```python
from build123d import *

# Parameters (mm, degrees)
SKETCH4_W          = 1.2
SKETCH4_H          = 1.2
CUT_EXTRUDE1_DEPTH = 50


with BuildPart() as part:
    # Sketch3 → Boss-Revolve (revolve)
    with BuildSketch(Plane.XY, mode=Mode.PRIVATE) as boss_revolve_sk:
        with BuildLine():
            Line((0, 0), (15, 0))
            Line((15, 0), (15, 2.5))
            Line((15, 2.5), (4.6, 2.5))
            Line((4.6, 2.5), (4.265, 2.165))
            Line((4.265, 2.165), (3.685, 2.165))
            ThreePointArc((3.685, 2.165), (3.200631855, 2.365631855), (3, 2.85))
            Line((3, 2.85), (3, 4.75))
            Line((3, 4.75), (1.369266386, 4.607329296))
            ThreePointArc((1.369266386, 4.607329296), (0.394083995, 4.12642256), (0, 3.113037248))
            Line((0, 3.113037248), (0, 0))
        make_face()
    revolve(boss_revolve_sk.sketch.rotate(Axis((-2.477021524, 0, 0), (1, 0, 0)), 90), axis=Axis((-2.477021524, 0, 0), (1, 0, 0)))

    # Sketch4 → Cut-Extrude1 (cut, symmetric)
    with BuildSketch(Plane.XY):
        with Locations((0.6, 0)):
            Rectangle(SKETCH4_W, SKETCH4_H)
    extrude(amount=CUT_EXTRUDE1_DEPTH, both=True, mode=Mode.SUBTRACT)

    # Sketch5 → Cut-Revolve1 (revolve, cut)
    with BuildSketch(Plane.XY, mode=Mode.PRIVATE) as cut_revolve1_sk:
        Polygon((14.595667195, 2.5), (15.395667195, 2.5), (15, 1.8072), align=None)
    revolve(cut_revolve1_sk.sketch.rotate(Axis((6.174994867, 0, 0), (-1, 0, 0)), 270), axis=Axis((6.174994867, 0, 0), (-1, 0, 0)), mode=Mode.SUBTRACT)


solid = part.part
```
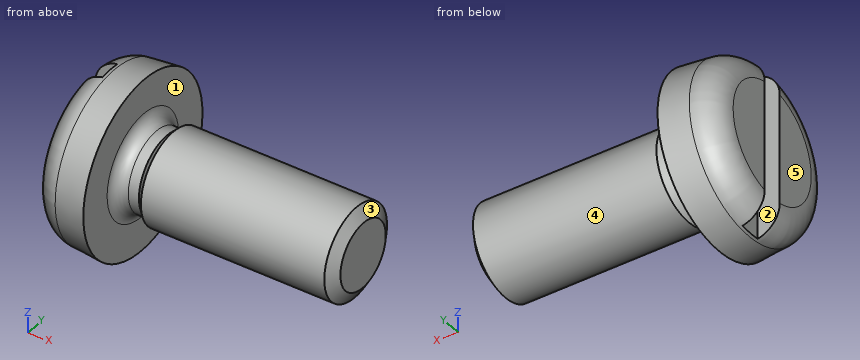
Work out the finished part from the listing and answer in its coordinate system (mm). Face numbers are marked on the shaded views. A direction names the side the tool comes from. Give positions to 0.01 mm unless a question says otherwise; leave off trailing zeros. Loops run counter-clockwise (first coordinate to the right, second up) from the corner with the lowest first, then second, coordinate; pieces in that order, holes last. Notation, with made-up numbers: (-13, -22) - (4, -22) arc R20 cw to (4, -7) - close; hole circle Ø2 at (23, 37). An arc over 180 degrees is marked (long way). Use CSV: the item, a comma, the result in double quotes. Start each with the question number.
(1) Find section A-A, the plane z = 0. Determine the outline of the cut face in (x, y) (3 decimals).
(2) Find section B-B, the plane y = 0. Determine the outline of the cut face in (x, z) (3 decimals).
(3) Determine the mould class of the marked faces 1, 2 and 3 for opening direction Y: released by +Y, released by -Y, zero draft, split by the parting line, or undercut.
(4) Each of these flat-tipped pins is pushed along its axis until it touches: pin 1 (3 mm diameter, centred on x = 7, y = -2, fed in from +Z); pin 2 (1.3 mm diameter, centred on x = 0.5, z = 2, fed in from -Y); pin 3 (1 mm diameter, centred on y = 0, z = 0, fed in from -X). Where does it stop, or does it pass through?
(5) Find the intervals of material crossed by L1, parallel to X at y = 2.5, z = -1.75; L2, parallel to Z at x = 2.25, y = 3.5; L3, parallel to X at y = -1.75, z = 4, in increasing order.
(6) Find section C-C, the plane x = 9. Determine the outline of the cut face in (y, z).
(7) A tool of negligible diameter and unlimited length cuts with its end or side. For the marked faces 4 and 5, from which of +Z, -Z, +X, -X, +Y, -Y can it reach the whole face along a straight path? Write none if from no direction.
Results found:
1,outline,"(0, -3.113) arc R1.5 ccw to (1.369, -4.607) - (3, -4.75) - (3, -2.85) arc R0.685 cw to (3.685, -2.165) - (4.265, -2.165) - (4.6, -2.5) - (14.596, -2.5) - (15, -1.807) - (15, 1.807) - (14.596, 2.5) - (4.6, 2.5) - (4.265, 2.165) - (3.685, 2.165) arc R0.685 cw to (3, 2.85) - (3, 4.75) - (1.369, 4.607) arc R1.5 ccw to (0, 3.113) - (0, 0.6) - (1.2, 0.6) - (1.2, -0.6) - (0, -0.6) - close"
2,outline,"(1.2, -4.583) arc R1.5 ccw to (1.369, -4.607) - (3, -4.75) - (3, -2.85) arc R0.685 cw to (3.685, -2.165) - (4.265, -2.165) - (4.6, -2.5) - (14.596, -2.5) - (15, -1.807) - (15, 1.807) - (14.596, 2.5) - (4.6, 2.5) - (4.265, 2.165) - (3.685, 2.165) arc R0.685 cw to (3, 2.85) - (3, 4.75) - (1.369, 4.607) arc R1.5 ccw to (1.2, 4.583) - close"
3,face 1,"zero draft"
3,face 2,"undercut"
3,face 3,"split by the parting line"
4,pin 1,"z = 2.45"
4,pin 2,"y = -4.24"
4,pin 3,"x = 1.2"
5,L1,"0 to 3"
5,L2,"-3.11 to 3.11"
5,L3,"0.68 to 3"
6,outline,"circle Ø5 at (0, 0)"
7,face 4,"+X"
7,face 5,"+Z, -Z, -X, +Y, -Y"
